The model under review builds one solid part; all positions refer to its coordinate system, in mm. Give positions to 0.01 mm unless a question says otherwise; leave off trailing zeros. Loops run counter-clockwise (first coordinate to the right, second up) from the corner with the lowest first, then second, coordinate; pieces in that order, holes last. Notation, with made-up numbers: (43, -28) - (64, -28) arc R34 cw to (64, 9) - close; hole circle Ø4 at (-36.75, 31). An arc over 180 degrees is marked (long way). Answer as a JSON object with one key per item and string values.
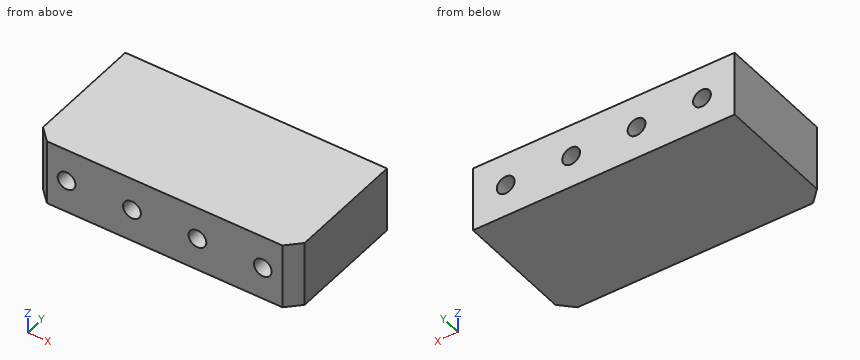
from build123d import *

# Parameters (mm, degrees)
SKETCH1_W           = 100
SKETCH1_H           = 50
BOSS_EXTRUDE1_DEPTH = 25
M8_TAPPED_HOLE1_D   = 6.8
CHAMFER1_SIZE       = 5


with BuildPart() as part:
    # Sketch1 → Boss-Extrude1 (new body)
    with BuildSketch(Plane.XY):
        Rectangle(SKETCH1_W, SKETCH1_H)
    extrude(amount=BOSS_EXTRUDE1_DEPTH)

    # M8 Tapped Hole1 (through all)
    with Locations(Plane(origin=(0, 25, 0), x_dir=(1, 0, 0), z_dir=(0, 1, 0))):
        with Locations((-37.5, -12.5), (-12.5, -12.5), (12.5, -12.5), (37.5, -12.5)):
            Hole(M8_TAPPED_HOLE1_D / 2)

    # Chamfer1
    chamfer1_edges = [part.edges().sort_by_distance(p)[0] for p in [
        (-50, -25, 12.5),
        (50, -25, 12.5),
    ]]
    chamfer(chamfer1_edges, length=CHAMFER1_SIZE)


solid = part.part
Q1. Consider section D-D, the plane x = -11.5. State the section outline as (y, z) points, plus the area to 3 significant figures.
Results:
{"outline": "(-25, 0) - (25, 0) - (25, 9.25) - (-25, 9.25) - close; (-25, 15.75) - (25, 15.75) - (25, 25) - (-25, 25) - close", "area": "925 mm^2"}
Q2. Consider section C-C, the plane z = 12.5. State the section outline as (x, y) points, plus the area to 4 significant figures.
Results:
{"outline": "(-50, -20) - (-45, -25) - (-40.9, -25) - (-40.9, 25) - (-50, 25) - close; (-34.1, -25) - (-15.9, -25) - (-15.9, 25) - (-34.1, 25) - close; (-9.1, -25) - (9.1, -25) - (9.1, 25) - (-9.1, 25) - close; (15.9, -25) - (34.1, -25) - (34.1, 25) - (15.9, 25) - close; (40.9, -25) - (45, -25) - (50, -20) - (50, 25) - (40.9, 25) - close", "area": "3,615 mm^2"}
Q3. To check wall thickness, follow probe 1 along X at (y, z) = (-2.5, 12.5); probe 2 along Z at (x, y) = (-12.5, 21.5); probe 3 along X at (y, z) = (17, 13.75). State the ranges of each line that lie inside material, in increasing order. Write a range as [from, to].
Results:
{"probe 1": "x = [-50, -40.9], [-34.1, -15.9], [-9.1, 9.1], [15.9, 34.1], [40.9, 50]", "probe 2": "z = [0, 9.1], [15.9, 25]", "probe 3": "x = [-50, -40.66], [-34.34, -15.66], [-9.34, 9.34], [15.66, 34.34], [40.66, 50]"}
Q4. Consider section A-A, the plane x = 12.5. State the section outline as (y, z) points, plus the area to 3 significant figures.
Results:
{"outline": "(-25, 0) - (25, 0) - (25, 9.1) - (-25, 9.1) - close; (-25, 15.9) - (25, 15.9) - (25, 25) - (-25, 25) - close", "area": "910 mm^2"}
Q5. Consider section B-B, the plane y = 8. State the section outline as (x, z) points, plus the area to 3 significant figures.
Results:
{"outline": "(-50, 0) - (50, 0) - (50, 25) - (-50, 25) - close; hole circle Ø6.8 at (-37.5, 12.5); hole circle Ø6.8 at (-12.5, 12.5); hole circle Ø6.8 at (12.5, 12.5); hole circle Ø6.8 at (37.5, 12.5)", "area": "2,350 mm^2"}
